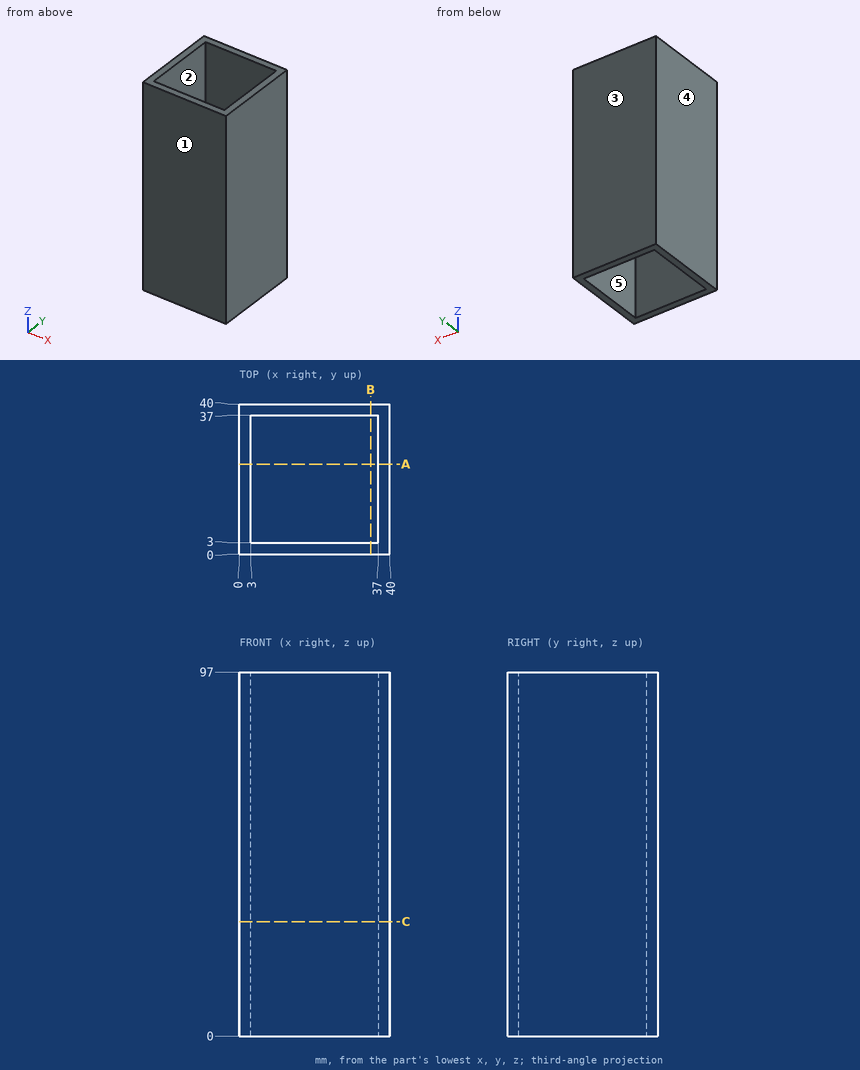
Input: dimensioned drawing with shaded views. Units: mm. Origin: part minimum x, y, z. A direction names the side the tool comes from. Give positions to 0.01 mm unless a question says otherwise; leave off trailing zeros. Loops run counter-clockwise (first coordinate to the right, second up) from the corner with the lowest first, then second, coordinate; pieces in that order, holes last. Notation, with made-up numbers: (6, 65) -> (19, 65) arc R21 cw to (19, 90) -> close; hole circle Ø1 at (-14.5, 52.25). An arc over 180 degrees is marked (long way). Return JSON: item names as keys, results as strings.
Item 1: Section A-A, the plane y = 24. Output: boundary loops of the cut face in (x, z), plus the area to 3 significant figures.
Filled in:
{"outline": "(0, 0) -> (3, 0) -> (3, 97) -> (0, 97) -> close; (37, 0) -> (40, 0) -> (40, 97) -> (37, 97) -> close", "area": "582 mm^2"}
Item 2: Section C-C, the plane z = 30.5. Output: boundary loops of the cut face in (x, y), plus the area to 3 significant figures.
Filled in:
{"outline": "(0, 0) -> (40, 0) -> (40, 40) -> (0, 40) -> close; hole (3, 3) -> (37, 3) -> (37, 37) -> (3, 37) -> close", "area": "444 mm^2"}
Item 3: Access query for the marked faces 1 and 2. Directions: +Z, -Z, +X, -X, +Y, -Y. A direction counts if a zero-diameter tool reaches every point of the face in a straight line with its end or side. Return the directions, or none.
Filled in:
{"face 1": "+Z, -Z, +X, -X, -Y", "face 2": "+Z, -Z"}
Item 4: Line query: line 1 (Y direction, x = 8.5, z = 37.5). Output: solid intervals per line, ascending.
Filled in:
{"line 1": "0 to 3, 37 to 40"}
Item 5: Mould query, pull axis X, two halves, no side actions, for the marked faces 3, 4 and 5. Classes: released by +X, released by -X, zero draft, split by the parting line, or undercut.
Filled in:
{"face 3": "zero draft", "face 4": "released by -X", "face 5": "undercut"}
